Check sheet for the modelled part. Datum: model origin and axes. Units: mm. A direction names the side the tool comes from. Coordinates: 2 decimals unless noted, no trailing zeros. Write each loop counter-clockwise with the first axis right and the second up, starting at its lowest first coordinate (ties: lowest second). Pieces come first, ordered by that corner, then holes. Notation, with made-up numbers: (85.5, 22) -> (128.5, 22) arc R24 cw to (128.5, 60) -> close; hole circle Ø7 at (-35, 74). An arc over 180 degrees is marked (long way). Put each result on its own line as item: value.
```python
from build123d import *

# Parameters (mm, degrees)
EXTRUDE_1_DEPTH              = 11
HOLE_WIZARD_M6_1_D           = 6.5
HOLE_WIZARD_M6_1_CBORE_D     = 11
HOLE_WIZARD_M6_1_CBORE_DEPTH = 30
CUT_EXTRUDE_1_DEPTH          = 20
CHAMFER_1_SIZE               = 1.5


with BuildPart() as part:
    # 草图1 → 凸台-拉伸1 (new, symmetric)
    with BuildSketch(Plane.XY):
        Polygon((-52.5, 0), (-36.5, 0), (-36.5, 26), (-33.5, 29), (33.5, 29), (36.5, 26), (36.5, 0), (52.5, 0), (52.5, 22), (37.5, 37), (-37.5, 37), (-52.5, 22), align=None)
    extrude(amount=EXTRUDE_1_DEPTH, both=True)

    # M6 六角凹头螺钉的柱形沉头孔1 (through all)
    with Locations(Plane(origin=(0, 37, 0), x_dir=(1, 0, 0), z_dir=(0, 1, 0))):
        with Locations((-45, 0), (45, 0)):
            CounterBoreHole(HOLE_WIZARD_M6_1_D / 2, HOLE_WIZARD_M6_1_CBORE_D / 2, HOLE_WIZARD_M6_1_CBORE_DEPTH)

    # 草图4 → 切除-拉伸1 (cut)
    with BuildSketch(Plane(origin=(0, 37, 0), x_dir=(1, 0, 0), z_dir=(0, 1, 0))):
        with BuildLine():
            Line((-52.5, 7), (-45, 7))
            ThreePointArc((-45, 7), (-38, 0), (-45, -7))
            Line((-45, -7), (-52.5, -7))
            ThreePointArc((-52.5, -7), (-59.5, 0), (-52.5, 7))
        make_face()
        with BuildLine():
            Line((52.5, 7), (45, 7))
            ThreePointArc((45, 7), (38, 0), (45, -7))
            Line((45, -7), (52.5, -7))
            ThreePointArc((52.5, -7), (59.5, 0), (52.5, 7))
        make_face()
    extrude(amount=-CUT_EXTRUDE_1_DEPTH, mode=Mode.SUBTRACT)

    # 倒角1
    chamfer_1_edges = [part.edges().sort_by_distance(p)[0] for p in [
        (-36.5, 13, 11),
        (-45, 29.5, -11),
        (0, 37, -11),
        (45, 29.5, -11),
        (52.5, 11, -11),
        (44.5, 0, -11),
        (36.5, 13, -11),
        (-35, 27.5, 11),
        (35, 27.5, -11),
        (0, 29, -11),
        (-35, 27.5, -11),
        (-36.5, 13, -11),
        (-44.5, 0, -11),
        (-52.5, 11, -11),
        (0, 29, 11),
        (35, 27.5, 11),
        (36.5, 13, 11),
        (44.5, 0, 11),
        (52.5, 11, 11),
        (45, 29.5, 11),
        (0, 37, 11),
        (-45, 29.5, 11),
        (-52.5, 11, 11),
        (-44.5, 0, 11),
    ]]
    chamfer(chamfer_1_edges, length=CHAMFER_1_SIZE)


solid = part.part
```
Q1. Tool access check on faces 5 (the cylindrical face through (-50.495, 12.07, -0.242)), 6 (the cylindrical face through (-38, 25, 0)), 7 (the flat face through (35, 27.5, 0.1)), 8 (the flat face through (48, 22, -7)), 9 (the flat face through (35.5, 28.05, 10.24)). Record the directions out of +Z, -Z, +X, -X, +Y, -Y that give a thin tool (end or side, any length) a straight path to the whole face; none if there is none.
Recorded:
face 5: +Y
face 6: -X, +Y
face 7: +Z, -Z, -Y
face 8: +X, +Y
face 9: +Z, -Y
Q2. Cross-section at B-B (z = 0). State how many separate pieces and enclosed holes the cut face has, plus the area to 3 significant figures.
Recorded:
separate pieces: 3
enclosed holes: 0
area: 886 mm2
Q3. Cross-section at A-A (y = 9.5). Record the cut outline in (x, z), plus the area to 3 significant figures.
Recorded:
outline: (-52.5, -9.5) -> (-51, -11) -> (-38, -11) -> (-36.5, -9.5) -> (-36.5, 9.5) -> (-38, 11) -> (-51, 11) -> (-52.5, 9.5) -> close; (36.5, -9.5) -> (38, -11) -> (51, -11) -> (52.5, -9.5) -> (52.5, 9.5) -> (51, 11) -> (38, 11) -> (36.5, 9.5) -> close; hole circle Ø11 at (-45, 0); hole circle Ø11 at (45, 0)
area: 505 mm2
Q4. Depth check by flat-ended pin: P1, Ø2, axis at x = -49.5, y = 24.5, coming from the -Z side; P2, Ø1.5, axis at x = 23, z = -4.5, coming from the -Y side; P3, Ø12, axis at x = 46, z = 0.5, coming from the +Y side; P4, Ø4, axis at x = 45, z = 0, coming from the -Y side. Enter the tip coordinate at first touch or a pass-through.
Recorded:
P1: stops at z = -10.85
P2: stops at y = 29
P3: stops at y = 17
P4: passes through
Q5. Material ranges on line 1 along Z through (x, y) = (45, 13.75); line 2 along X through (y, z) = (4, -9); line 3 along Z through (x, y) = (-45, 3), recorded low to high.
Recorded:
line 1: z = -11 to -5.5, 5.5 to 11
line 2: x = -52.5 to -36.5, 36.5 to 52.5
line 3: z = -11 to -3.25, 3.25 to 11
Q6. Mould release check, pull along Z, two halves, no side actions. Record for faces 1 (the flat face through (44.58, 28.87, -10.24)), 2 (the flat face through (49, 7, 0)), 3 (the flat face through (50, 17, 3)), 4 (the flat face through (-36.5, 13, 0)): released by +Z, released by -Z, zero draft, split by the parting line, or undercut.
Recorded:
face 1: released by -Z
face 2: undercut
face 3: undercut
face 4: zero draft
Q7. Cross-section at C-C (y = 24.5). Record the cut outline in (x, z).
Recorded:
outline: (-50, -9.5) -> (-47.88, -11) -> (-38, -11) -> (-36.5, -9.5) -> (-36.5, 9.5) -> (-38, 11) -> (-47.88, 11) -> (-50, 9.5) -> (-50, 7) -> (-45, 7) arc R7 cw to (-45, -7) -> (-50, -7) -> close; (36.5, -9.5) -> (38, -11) -> (47.88, -11) -> (50, -9.5) -> (50, -7) -> (45, -7) arc R7 cw to (45, 7) -> (50, 7) -> (50, 9.5) -> (47.88, 11) -> (38, 11) -> (36.5, 9.5) -> close
Q8. Cross-section at D-D (x = 8.5). Record the cut outline in (y, z).
Recorded:
outline: (29, -9.5) -> (30.5, -11) -> (35.5, -11) -> (37, -9.5) -> (37, 9.5) -> (35.5, 11) -> (30.5, 11) -> (29, 9.5) -> close
